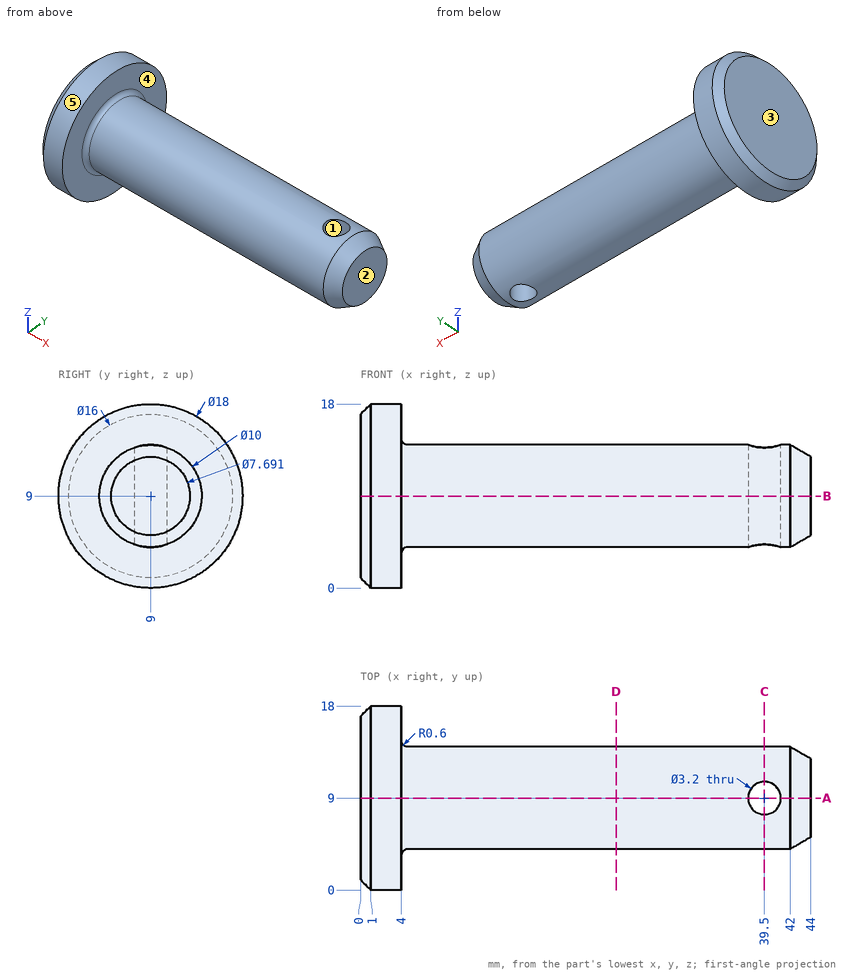
Could you check a few things on this drawing? It's one solid part, dimensions in mm from its lowest x, y, z. A direction names the side the tool comes from. Round coordinates to 2 decimals unless told otherwise and drop trailing zeros. Order: outer loops, then holes, each group sorted by start corner. A loop starts at its lowest first (then second) coordinate and runs counter-clockwise, first axis right, second up. Notation, with made-up numbers: (25, -6.75) -> (50, -6.75) arc R11 ccw to (50, 4.25) -> close; hole circle Ø11 at (75.5, 31). An arc over 180 degrees is marked (long way). One line per question, with ' | ' between items.
Q1. If I drill on line 1 (X direction, y = 9, z = 8.5); line 2 (Y direction, x = 39.5, z = 9); line 3 (X direction, y = 2.25, z = 10.5), over which ranges is the centre line in solid material (lowest first)? Write a range as from..to.
Computed values:
line 1: 0..37.9, 41.1..44 | line 2: 4..7.4, 10.6..14 | line 3: 0..4
Q2. If we section it at B-B on z = 9: Write out the boundary of the cut face in (x, y) (1 decimal), plus the area to 3 significant figures.
Computed values:
outline: (0, 1) -> (1, 0) -> (4, 0) -> (4, 3.4) arc R0.6 cw to (4.6, 4) -> (42, 4) -> (44, 5.2) -> (44, 12.8) -> (42, 14) -> (4.6, 14) arc R0.6 cw to (4, 14.6) -> (4, 18) -> (1, 18) -> (0, 17) -> close; hole circle Ø3.2 at (39.5, 9) | area: 461 mm²
Q3. If we section it at D-D on x = 25: Write out the boundary of the cut face in (y, z).
Computed values:
outline: circle Ø10 at (9, 9)
Q4. If we section it at C-C on x = 39.5: Write out the boundary of the cut face in (y, z).
Computed values:
outline: (7.4, 4.26) -> (7.4, 13.74) arc R5 ccw to start; (10.6, 4.26) arc R5 ccw to (10.6, 13.74) -> close
Q5. If we section it at A-A on y = 9: Write out the boundary of the cut face in (x, z) (1 decimal).
Computed values:
outline: (0, 1) -> (1, 0) -> (4, 0) -> (4, 3.4) arc R0.6 cw to (4.6, 4) -> (37.9, 4) -> (37.9, 14) -> (4.6, 14) arc R0.6 cw to (4, 14.6) -> (4, 18) -> (1, 18) -> (0, 17) -> close; (41.1, 4) -> (42, 4) -> (44, 5.2) -> (44, 12.8) -> (42, 14) -> (41.1, 14) -> close
Q6. Which directions (+Z, -Z, +X, -X, +Y, -Y) give clear straight access to the entire face, cutting with the end or side of a thin tool? Please do the marked faces 4 and 5.
Computed values:
face 4: +X | face 5: +X, -X
Q7. I'm going to push flat-ended pins straight in: pin 1 (4 mm diameter, centred on x = 11, y = 14.5, fed in from +Z); pin 2 (6 mm diameter, centred on x = 32, y = 11.5, fed in from -Z); pin 3 (3 mm diameter, centred on x = 10, z = 2, fed in from -Y); pin 4 (1.5 mm diameter, centred on y = 5.5, z = 5.5, fed in from +X) (1 decimal). Where does each tip first touch, or does it pass through?
Computed values:
pin 1: z = 12.57 | pin 2: z = 4 | pin 3: through | pin 4: x = 43.4
Q8. We'd pull the mould along X, two halves only. Please class the marked faces 1, 2 and 3: released by +X, released by -X, zero draft, split by the parting line, or undercut.
Computed values:
face 1: undercut | face 2: released by +X | face 3: released by -X
